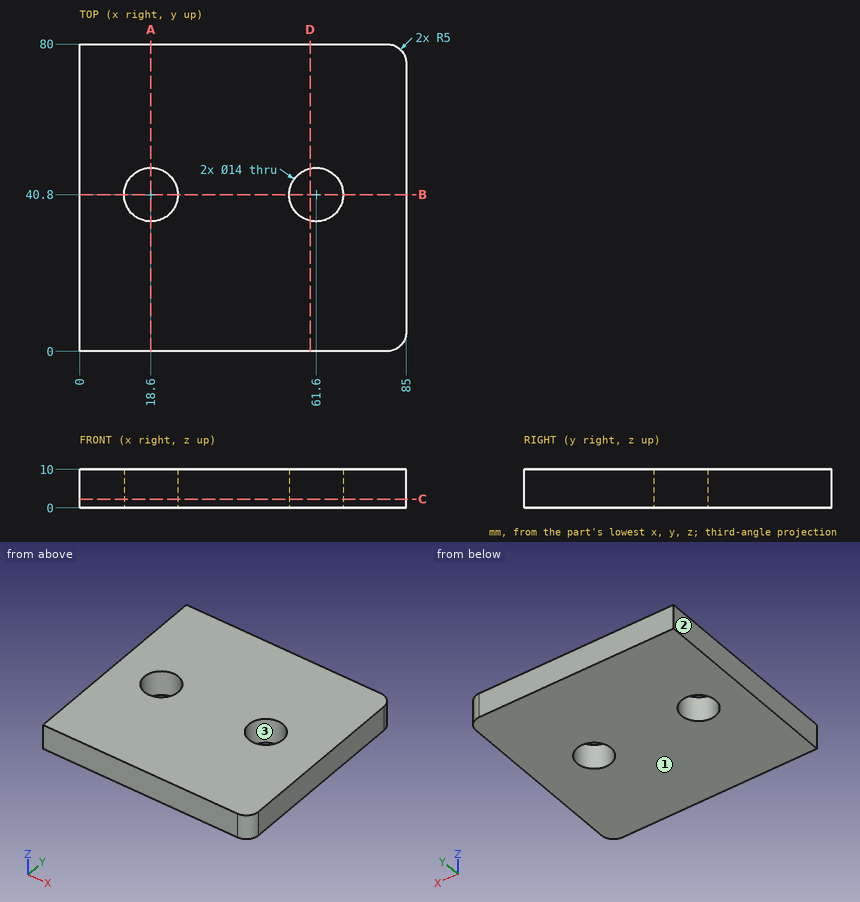
Could you check a few things on this drawing? It's one solid part, dimensions in mm from its lowest x, y, z. Coordinates: 2 decimals unless noted, no trailing zeros. Order: outer loops, then holes, each group sorted by start corner. A loop starts at its lowest first (then second) coordinate and runs counter-clockwise, first axis right, second up. Notation, with made-up numbers: M 64.25,-16 L 114.25,-16 A26 ccw 114.25,7 Z; hole C 82.25,-29.5 d6. An arc over 180 degrees is marked long. Use one line per item in the form item = value. Start each with the question number.
1. Suppose I cut it at D-D on x = 60. Write out the boundary of the cut face in (y, z).
2. Suppose I cut it at C-C on z = 2.25. Write out the boundary of the cut face in (x, y), then the cut area to 3 significant figures.
3. For pin 1 (12.5 mm diameter, centred on x = 61.6, y = 40.8, fed in from +Z), with a flat end and sliding along its axis, tell me the tip position at first contact or that it passes through.
4. Suppose I cut it at A-A on x = 18.6. Write out the boundary of the cut face in (y, z).
5. Please list where these lines run through material, in increasing order: line 1 (Y direction, x = 18.6, z = 7.5); line 2 (Y direction, x = 64, z = 8.5); line 3 (Y direction, x = 81, z = 8.5).
6. We'd pull the mould along X, two halves only. Please class the marked faces 1, 2 and 3: +X half, -X half, draft (parallel to the pull), parting line (faces both ways), or undercut.
7. Suppose I cut it at B-B on y = 40.8. Write out the boundary of the cut face in (x, z), then the cut area to 3 significant figures.
Geometry says:
q1.outline = M 0,0 L 33.99,0 L 33.99,10 L 0,10 Z; M 47.61,0 L 80,0 L 80,10 L 47.61,10 Z
q2.outline = M 0,0 L 80,0 A5 ccw 85,5 L 85,75 A5 ccw 80,80 L 0,80 Z; hole C 18.6,40.8 d14; hole C 61.6,40.8 d14
q2.area = 6,480 mm^2
q3.pin_1 = through
q4.outline = M 0,0 L 33.8,0 L 33.8,10 L 0,10 Z; M 47.8,0 L 80,0 L 80,10 L 47.8,10 Z
q5.line_1 = 0 to 33.8, 47.8 to 80
q5.line_2 = 0 to 34.22, 47.38 to 80
q5.line_3 = 0.1 to 79.9
q6.face_1 = draft
q6.face_2 = -X half
q6.face_3 = undercut
q7.outline = M 0,0 L 11.6,0 L 11.6,10 L 0,10 Z; M 25.6,0 L 54.6,0 L 54.6,10 L 25.6,10 Z; M 68.6,0 L 85,0 L 85,10 L 68.6,10 Z
q7.area = 570 mm^2
